```python
from build123d import *

# Parameters (mm, degrees)
SKETCH_1_W          = 80
SKETCH_1_H          = 30
EXTRUDE_1_DEPTH     = 10
SKETCH_2_R          = 1.25
CUT_EXTRUDE_1_DEPTH = 2


with BuildPart() as part:
    # 草图1 → 凸台-拉伸1 (new body)
    with BuildSketch(Plane.XY):
        Rectangle(SKETCH_1_W, SKETCH_1_H)
    extrude(amount=EXTRUDE_1_DEPTH)

    # 草图2 → 切除-拉伸1 (cut)
    with BuildSketch(Plane.XY.offset(10)):
        with Locations((-10, 0)):
            Circle(SKETCH_2_R)
        with Locations((10, 0)):
            Circle(SKETCH_2_R)
    extrude(amount=-CUT_EXTRUDE_1_DEPTH, mode=Mode.SUBTRACT)


solid = part.part
```
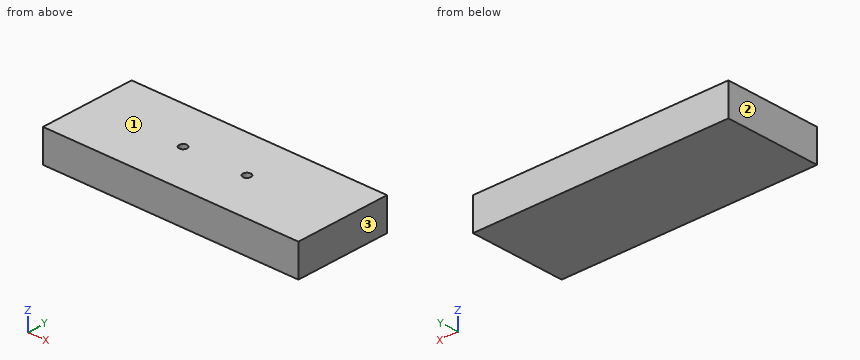
Geometry check sheet. Reference: the model listing, model coordinates, mm. Face numbers are marked on the shaded views. Round coordinates to 2 decimals unless told otherwise and drop trailing zeros. Order: outer loops, then holes, each group sorted by start corner. A loop starts at its lowest first (then second) coordinate and runs counter-clockwise, first axis right, second up. Notation, with made-up numbers: (60, 63.5) -> (87, 63.5) arc R17 cw to (87, 94.5) -> close; hole circle Ø5 at (7, -23). An arc over 180 degrees is marked (long way). Return JSON: item names as keys, results as strings. Group by question number.
Q1. Section check A-A, the plane x = -10. Record the boundary of the cut face in (y, z), plus the area to 3 significant figures.
Q2. Material ranges on probe 1 along Y at (x, z) = (10, 9.35), recorded low to high. Write a range as from..to.
Q3. Release check for a two-part mould opening along X. For the marked faces 1, 2 and 3 record: released by +X, released by -X, zero draft, split by the parting line, or undercut.
Q4. Gauge pin test, flat end, axial feed: pin 1 (0.8 mm diameter, centred on x = -10.5, y = -0.5, fed in from +Z). Record the tip position at first contact, or that the pin passes through.
Numbers:
{
 "1": {"outline": "(-15, 0) -> (15, 0) -> (15, 10) -> (1.25, 10) -> (1.25, 8) -> (-1.25, 8) -> (-1.25, 10) -> (-15, 10) -> close", "area": "295 mm^2"},
 "2": {"probe 1": "-15..-1.25, 1.25..15"},
 "3": {"face 1": "zero draft", "face 2": "released by -X", "face 3": "released by +X"},
 "4": {"pin 1": "z = 8"}
}
